Could you check a few things on this model? Use its own coordinates, in mm. A direction names the side the tool comes from. Round coordinates to 2 decimals unless told otherwise and drop trailing zeros. Write each loop counter-clockwise with the first axis right and the second up, starting at its lowest first coordinate (ties: lowest second). Pieces come first, ordered by that corner, then holes. Notation, with made-up numbers: M 85.25,-32.5 L 122.25,-32.5 A20 cw 122.25,-1.5 Z; hole C 27,15 d5. An arc over 180 degrees is marked long. One line per item, written item: value. Start each with the question number.
(1) I want a section at C-C on z = -671.5. Please give me the cut outline in (x, y), and give its area (3 significant figures).
(2) Thinking about a two-plate mould opening in Y: for faces 3 (the face through (0, 40.5, 13)), 4 (the face through (40.5, 0, 13)), 5 (the face through (0, -40.5, 13)), 6 (the face through (36.5, 0, 13)), which applies, released by +Y, released by -Y, zero draft, split by the parting line, or undercut?
(3) Which directions (+Z, -Z, +X, -X, +Y, -Y) give clear straight access to the entire face, cutting with the end or side of a thin tool? Please do faces 1 (the face through (0, 36.5, 13)), 2 (the face through (-40.5, 0, 13)).
(4) I want a section at A-A on x = -11.5. Please give me the cut outline in (y, z), and give its area (3 significant figures).
(5) If I drill on L1, parallel to Y at x = -19, z = -323; L2, parallel to Y at x = -36, z = -490, over which ranges is the centre line in solid material (lowest first)?
```python
from build123d import *

# Parameters (mm, degrees)
BOSS_EXTRUDE_1_DEPTH = 905.5


with BuildPart() as part:
    # Sketch 1 → Boss-Extrude 1 (new, symmetric)
    with BuildSketch(Plane.XY):
        with BuildLine():
            Line((0, 40.5), (-34.5, 40.5))
            ThreePointArc((-34.5, 40.5), (-38.742640687, 38.742640687), (-40.5, 34.5))
            Line((-40.5, 34.5), (-40.5, 0))
            Line((-40.5, 0), (-40.5, -34.5))
            ThreePointArc((-40.5, -34.5), (-38.742640687, -38.742640687), (-34.5, -40.5))
            Line((-34.5, -40.5), (34.5, -40.5))
            ThreePointArc((34.5, -40.5), (38.742640687, -38.742640687), (40.5, -34.5))
            Line((40.5, -34.5), (40.5, 0))
            Line((40.5, 0), (40.5, 34.5))
            ThreePointArc((40.5, 34.5), (38.742640687, 38.742640687), (34.5, 40.5))
            Line((34.5, 40.5), (0, 40.5))
        make_face()
        with BuildLine():
            Line((0, 36.5), (-34.5, 36.5))
            ThreePointArc((-34.5, 36.5), (-35.914213562, 35.914213562), (-36.5, 34.5))
            Line((-36.5, 34.5), (-36.5, 0))
            Line((-36.5, 0), (-36.5, -34.5))
            ThreePointArc((-36.5, -34.5), (-35.914213562, -35.914213562), (-34.5, -36.5))
            Line((-34.5, -36.5), (34.5, -36.5))
            ThreePointArc((34.5, -36.5), (35.914213562, -35.914213562), (36.5, -34.5))
            Line((36.5, -34.5), (36.5, 0))
            Line((36.5, 0), (36.5, 34.5))
            ThreePointArc((36.5, 34.5), (35.914213562, 35.914213562), (34.5, 36.5))
            Line((34.5, 36.5), (0, 36.5))
        make_face(mode=Mode.SUBTRACT)
    extrude(amount=BOSS_EXTRUDE_1_DEPTH, both=True)


solid = part.part
```
Found:
1. outline: M -40.5,-34.5 A6 ccw -34.5,-40.5 L 34.5,-40.5 A6 ccw 40.5,-34.5 L 40.5,34.5 A6 ccw 34.5,40.5 L -34.5,40.5 A6 ccw -40.5,34.5 Z; hole M -36.5,-34.5 A2 ccw -34.5,-36.5 L 34.5,-36.5 A2 ccw 36.5,-34.5 L 36.5,34.5 A2 ccw 34.5,36.5 L -34.5,36.5 A2 ccw -36.5,34.5 Z
1. area: 1,200 mm²
2. face 3: released by +Y
2. face 4: zero draft
2. face 5: released by -Y
2. face 6: undercut
3. face 1: +Z, -Z
3. face 2: +Z, -Z, -X, +Y, -Y
4. outline: M -40.5,-905.5 L -36.5,-905.5 L -36.5,905.5 L -40.5,905.5 Z; M 36.5,-905.5 L 40.5,-905.5 L 40.5,905.5 L 36.5,905.5 Z
4. area: 14,500 mm²
5. L1: y = -40.5 to -36.5, 36.5 to 40.5
5. L2: y = -40.31 to -35.82, 35.82 to 40.31
